Work out the finished part from the listing and answer in its coordinate system (mm). Face numbers are marked on the shaded views. Give positions to 0.01 mm unless a question says otherwise; leave off trailing zeros. Loops run counter-clockwise (first coordinate to the right, second up) from the corner with the lowest first, then second, coordinate; pieces in that order, holes last. Notation, with made-up numbers: M 65.5,60.5 L 86.5,60.5 A26 cw 86.5,82.5 Z; hole C -34.75,66 d5. An arc over 180 degrees is marked long. Write item = value, one per line. Start each with the question number.
1. Section C-C on x = -518.5 is taken. Determine the outline of the cut face in (y, z), plus the area to 3 significant figures.
2. Section A-A on z = 40 is taken. Determine the outline of the cut face in (x, y).
3. A flat-ended cylindrical pin translates along its axis: pin 1 Ø5 at (x, y) = (137.5, -54) entering from +Z. Find the tip coordinate at first contact, or state that the pin passes through.
4. The mould has two halves that part along Y. Classify the marked faces 1 and 2: released by +Y, released by -Y, zero draft, split by the parting line, or undercut.
5. Consider L1, parallel to Y at x = -744, z = 76; L2, parallel to X at y = -327, z = 62; L3, parallel to Z at x = -117, y = 610. Determine where each line is inside the solid, lowest interval first. Write a range as [from, to].
6. Section B-B on y = 367.5 is taken. Determine the outline of the cut face in (x, z), plus the area to 3 significant figures.
```python
from build123d import *

# Parameters (mm, degrees)
SKETCH1_W           = 1650
SKETCH1_H           = 1700
BOSS_EXTRUDE1_DEPTH = 80
SHELL1_T            = -2.3
CUT_EXTRUDE1_DEPTH  = 1892.302461268


with BuildPart() as part:
    # Sketch1 → Boss-Extrude1 (new body)
    with BuildSketch(Plane.XY):
        Rectangle(SKETCH1_W, SKETCH1_H)
    extrude(amount=BOSS_EXTRUDE1_DEPTH)

    # Shell1
    shell1_openings = [part.faces().sort_by_distance(p)[0] for p in [
        (0, 0, 80),
    ]]
    offset(amount=SHELL1_T, openings=shell1_openings, kind=Kind.INTERSECTION)

    # Sketch2 → Cut-Extrude1 (cut, through all)
    with BuildSketch(Plane.XZ.offset(850)):
        with BuildLine():
            Line((-785, 60), (-765, 60))
            ThreePointArc((-765, 60), (-745, 40), (-765, 20))
            Line((-765, 20), (-785, 20))
            ThreePointArc((-785, 20), (-805, 40), (-785, 60))
        make_face()
        with BuildLine():
            Line((785, 60), (765, 60))
            ThreePointArc((765, 60), (745, 40), (765, 20))
            Line((765, 20), (785, 20))
            ThreePointArc((785, 20), (805, 40), (785, 60))
        make_face()
    extrude(amount=-CUT_EXTRUDE1_DEPTH, mode=Mode.SUBTRACT)


solid = part.part
```
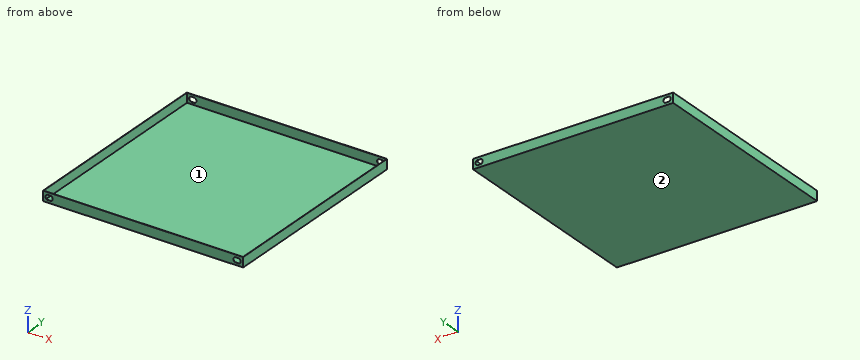
Verdict:
q1.outline = M -850,0 L 850,0 L 850,80 L 847.7,80 L 847.7,2.3 L -847.7,2.3 L -847.7,80 L -850,80 Z
q1.area = 4,270 mm2
q2.outline = M -825,-850 L -805,-850 L -805,-847.7 L -822.7,-847.7 L -822.7,847.7 L -805,847.7 L -805,850 L -825,850 Z; M -745,-850 L 745,-850 L 745,-847.7 L -745,-847.7 Z; M -745,847.7 L 745,847.7 L 745,850 L -745,850 Z; M 805,-850 L 825,-850 L 825,850 L 805,850 L 805,847.7 L 822.7,847.7 L 822.7,-847.7 L 805,-847.7 Z
q3.pin_1 = 2.3
q4.face_1 = undercut
q4.face_2 = zero draft
q5.L1 = [-850, -847.7], [847.7, 850]
q5.L2 = [-825, -822.7], [822.7, 825]
q5.L3 = [0, 2.3]
q6.outline = M -825,0 L 825,0 L 825,80 L 822.7,80 L 822.7,2.3 L -822.7,2.3 L -822.7,80 L -825,80 Z
q6.area = 4,150 mm2
